from build123d import *

# Parameters (mm, degrees)
HEAD_SLOT_CUT_DEPTH      = 72.232015274
HEAD_SLOT_CUT_DEPTH_BACK = 72.232015274
HEAD_SLOT_SKETCH_W       = 3
HEAD_SLOT_SKETCH_H       = 7
TRIM_CUT_1_DEPTH         = 72.216220063
TRIM_CUT_1_DEPTH_BACK    = 72.216220063
TRIM_CUT_1_SKETCH_W      = 30.281079354
TRIM_CUT_1_SKETCH_H      = 4.498315547
TRIM_CUT_2_DEPTH         = 66.899626103
TRIM_CUT_2_DEPTH_BACK    = 66.899626103
TRIM_CUT_2_SKETCH_W      = 29.08434912
TRIM_CUT_2_SKETCH_H      = 20.204065749


with BuildPart() as part:
    # Screw Half Profile Sketch → Screw Body Revolve (revolve)
    with BuildSketch(Plane.XY, mode=Mode.PRIVATE) as screw_body_revolve_sk:
        Polygon((0, 0), (5, 0), (5, 50), (15, 68), (0, 68), align=None)
    revolve(screw_body_revolve_sk.sketch.rotate(Axis((0, 68, 0), (0, -1, 0)), 180), axis=Axis((0, 68, 0), (0, -1, 0)))

    # Head Slot Sketch → Head Slot Cut (cut, two sides: drawn at the far end of the back side and taken through both)
    with BuildSketch(Plane.XY.offset(-HEAD_SLOT_CUT_DEPTH_BACK)):
        with Locations((0, 64.5)):
            Rectangle(HEAD_SLOT_SKETCH_W, HEAD_SLOT_SKETCH_H)
    extrude(amount=HEAD_SLOT_CUT_DEPTH + HEAD_SLOT_CUT_DEPTH_BACK, mode=Mode.SUBTRACT)

    # Trim Cut 1 Sketch → Trim Cut 1 (cut, two sides: drawn at the far end of the back side and taken through both)
    with BuildSketch(Plane.XY.offset(-TRIM_CUT_1_DEPTH_BACK)):
        with Locations((0.140539677, 65.750842226)):
            Rectangle(TRIM_CUT_1_SKETCH_W, TRIM_CUT_1_SKETCH_H)
    extrude(amount=TRIM_CUT_1_DEPTH + TRIM_CUT_1_DEPTH_BACK, mode=Mode.SUBTRACT)

    # Trim Cut 2 Sketch → Trim Cut 2 (cut, two sides: drawn at the far end of the back side and taken through both)
    with BuildSketch(Plane.XY.offset(-TRIM_CUT_2_DEPTH_BACK)):
        with Locations((-3.623465422, 10.102032875)):
            Rectangle(TRIM_CUT_2_SKETCH_W, TRIM_CUT_2_SKETCH_H)
    extrude(amount=TRIM_CUT_2_DEPTH + TRIM_CUT_2_DEPTH_BACK, mode=Mode.SUBTRACT)


solid = part.part
Geometry check sheet. Reference: the model listing, model coordinates, mm. A direction names the side the tool comes from. Round coordinates to 2 decimals unless told otherwise and drop trailing zeros. Loops run counter-clockwise (first coordinate to the right, second up) from the corner with the lowest first, then second, coordinate; pieces in that order, holes last. Notation, with made-up numbers: (44.5, 54.5) - (63.5, 54.5) arc R29 cw to (63.5, 88.5) - close; hole circle Ø8 at (54.5, 0). An arc over 180 degrees is marked (long way). One line per question, with ' | ' between items. Start each with the question number.
1. Draft check along X on faces 3 (the face through (0, 61, 0)), 4 (the face through (6, 63.502, 0)), 5 (the face through (5, 35, 0)). Enter one of: released by +X, released by -X, zero draft, split by the parting line, or undercut.
2. Cross-section at A-A on z = 0. Record the cut outline in (x, y), then the cut area to 3 significant figures.
3. Scan lines: line 1 (X direction, y = 36.5, z = -1); line 2 (Y direction, x = -5.5, z = 7.75); line 3 (Y direction, x = -4.25, z = -6.25). Record each from-to range of solid material in increasing order. Write a range as [from, to].
4. Tool access check on faces 1 (the face through (-1.5, 62, 0)), 2 (the face through (-6, 63.502, 0)). Record the directions out of +Z, -Z, +X, -X, +Y, -Y that give a thin tool (end or side, any length) a straight path to the whole face; none if there is none.
5. Cross-section at C-C on y = 34. Record the cut outline in (x, z).
6. Depth check by flat-ended pin: pin 1 (8 mm diameter, centred on x = 8.5, y = 29, fed in from -Z); pin 2 (0.8 mm diameter, centred on y = 62, z = -5, fed in from +X); pin 3 (6 mm diameter, centred on x = -5, y = 56, fed in from +Z). Enter the tip coordinate at first touch or a pass-through.
7. Cross-section at B-B on x = 0. Record the cut outline in (y, z), then the cut area to 3 significant figures.
Taken from the geometry:
1) face 3: undercut | face 4: zero draft | face 5: split by the parting line
2) outline: (-12.5, 63.5) - (-5, 50) - (-5, 20.2) - (5, 20.2) - (5, 50) - (12.5, 63.5) - (1.5, 63.5) - (1.5, 61) - (-1.5, 61) - (-1.5, 63.5) - close | area: 527 mm²
3) line 1: [-4.9, 4.9] | line 2: [58.11, 63.5] | line 3: [54.6, 63.5]
4) face 1: +Z, -Z, +Y | face 2: +Z, -Z, +X, -X, +Y
5) outline: circle Ø10 at (0, 0)
6) pin 1: z = -2.18 | pin 2: x = 10.85 | pin 3: z = 9.13
7) outline: (20.2, -5) - (50, -5) - (61, -11.11) - (61, 11.11) - (50, 5) - (20.2, 5) - close | area: 475 mm²
